The listing builds one solid part. Answer for the finished solid, in the listing's coordinates (mm). Face numbers are marked on the shaded views. A direction names the side the tool comes from. Coordinates: 2 decimals unless noted, no trailing zeros. Write each loop counter-clockwise with the first axis right and the second up, starting at its lowest first coordinate (ties: lowest second). Pieces come first, ordered by that corner, then holes.
```python
from build123d import *

# Parameters (mm, degrees)
SKETCH1_R           = 7.5
BOSS_EXTRUDE1_DEPTH = 40
SKETCH2_R           = 11.5
BOSS_EXTRUDE2_DEPTH = 13
CUT_EXTRUDE1_DEPTH  = 8


with BuildPart() as part:
    # Sketch1 → Boss-Extrude1 (new body)
    with BuildSketch(Plane.XY):
        Circle(SKETCH1_R)
    extrude(amount=BOSS_EXTRUDE1_DEPTH)

    # Sketch2 → Boss-Extrude2 (add)
    with BuildSketch(Plane.XY.offset(40)):
        with Locations(Location((0, 0, 0), (0, 0, 180))):
            Circle(SKETCH2_R)
    extrude(amount=BOSS_EXTRUDE2_DEPTH)

    # Sketch3 → Cut-Extrude1 (cut)
    with BuildSketch(Plane.XY.offset(53)):
        Polygon((6.412132048, -4.047977261), (6.711717166, 3.529080616), (0.299585118, 7.577057877), (-6.412132048, 4.047977261), (-6.711717166, -3.529080616), (-0.299585118, -7.577057877), align=None)
    extrude(amount=-CUT_EXTRUDE1_DEPTH, mode=Mode.SUBTRACT)


solid = part.part
```
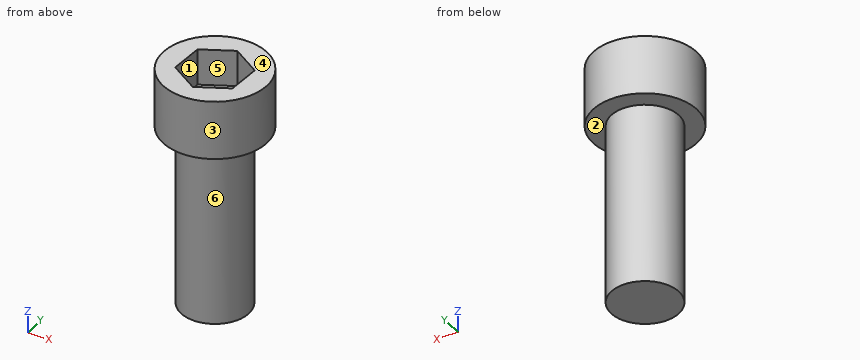
(1) Section D-D, the plane z = 14 is taken. Write down the section's boundary in (x, y), plus the area to 3 significant figures.
(2) Section C-C, the plane y = 6 is taken. Write down the section's boundary in (x, z), plus the area to 3 significant figures.
(3) Each of these flat-tipped pins is pushed along its axis until it touches: pin 1 (10 mm diameter, centred on y = 1, z = 18, fed in from +X); pin 2 (5 mm diameter, centred on y = -3.5, z = 30.5, fed in from -X); pin 3 (6 mm diameter, centred on x = -9, z = 12, fed in from +Y). Where does it stop, or does it pass through?
(4) Which of the six approach directions +Z, -Z, +X, -X, +Y, -Y give full straight-line access (tool end or side, diameter ignored) to the marked faces 1, 2 and 3?
(5) Section B-B, the plane z = 42.5 is taken. Write down the section's boundary in (x, y), plus the area to 3 significant figures.
(6) For a pull along Y with two mould halves and no side action, classify the marked faces 4, 5 and 6 as pulls with the +Y half, pulls with the -Y half, needs draft (parallel to the pull), parting line crosses it, or undercut.
(7) Find the intervals of material crossed by probe 1 along Z at (x, y) = (0.5, -0.25); probe 2 along Z at (x, y) = (9, 6.5); probe 3 along Y at (x, z) = (-1.75, 47), in increasing order.
(8) Section A-A, the plane x = 5.5 is taken. Write down the section's boundary in (y, z).
Solution:
1. outline: circle Ø15 at (0, 0)
1. area: 177 mm2
2. outline: (-9.81, 40) - (-4.5, 40) - (-4.5, 0) - (4.5, 0) - (4.5, 40) - (9.81, 40) - (9.81, 53) - (2.8, 53) - (2.8, 45) - (-2.7, 45) - (-2.7, 53) - (-9.81, 53) - close
2. area: 571 mm2
3. pin 1: stops at x = 7.5
3. pin 2: stops at x = -7.43
3. pin 3: stops at y = 4.5
4. face 1: +Z
4. face 2: -Z
4. face 3: +Z, -Z
5. outline: circle Ø23 at (0, 0)
5. area: 415 mm2
6. face 4: needs draft
6. face 5: undercut
6. face 6: parting line crosses it
7. probe 1: z = 0 to 45
7. probe 2: z = 40 to 53
7. probe 3: y = -11.37 to -6.66, 6.5 to 11.37
8. outline: (-10.1, 40) - (-5.1, 40) - (-5.1, 0) - (5.1, 0) - (5.1, 40) - (10.1, 40) - (10.1, 53) - (4.29, 53) - (4.29, 45) - (-4.53, 45) - (-4.53, 53) - (-10.1, 53) - close
